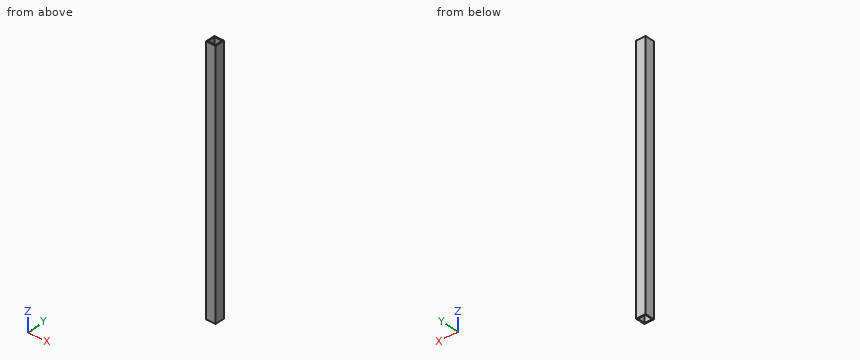
from build123d import *

# Parameters (mm, degrees)
SKETCH1_W           = 30
SKETCH1_H           = 30
SKETCH1_W_2         = 24
SKETCH1_H_2         = 24
BOSS_EXTRUDE2_DEPTH = 784


with BuildPart() as part:
    # Sketch1 → Boss-Extrude2 (new body)
    with BuildSketch(Plane.XY):
        with Locations((-1.115384615, 0.846363591)):
            Rectangle(SKETCH1_W, SKETCH1_H)
        with Locations((-1.115384615, 0.846363591)):
            Rectangle(SKETCH1_W_2, SKETCH1_H_2, mode=Mode.SUBTRACT)
    extrude(amount=BOSS_EXTRUDE2_DEPTH)


solid = part.part
Build history of the part. All positions in model axes, mm. Coordinates: 2 decimals unless noted, no trailing zeros. Write each loop counter-clockwise with the first axis right and the second up, starting at its lowest first coordinate (ties: lowest second). Pieces come first, ordered by that corner, then holes.
(1) Cut at A-A on y = 5.5. List the corners of the cut face in (x, z).
(2) Drill centre lines: line 1 (X direction, y = 0, z = 67); line 2 (Y direction, x = -0.25, z = 61.5). Where is each one in solid material? Low to high.
(3) Pin check, flat tips, straight feed: pin 1 Ø1.5 at (x, y) = (-6, -8.5) entering from -Z; pin 2 Ø12 at (x, y) = (2, 8.5) entering from -Z. Stop position of each tip, or through.
(4) Cut at B-B on x = -1.25. List the corners of the cut face in (y, z).
(5) Cut at C-C on z = 507. List the corners of the cut face in (x, y).
Working result:
1. outline: (-16.12, 0) - (-13.12, 0) - (-13.12, 784) - (-16.12, 784) - close; (10.88, 0) - (13.88, 0) - (13.88, 784) - (10.88, 784) - close
2. line 1: x = -16.12 to -13.12, 10.88 to 13.88
2. line 2: y = -14.15 to -11.15, 12.85 to 15.85
3. pin 1: passes through
3. pin 2: stops at z = 0
4. outline: (-14.15, 0) - (-11.15, 0) - (-11.15, 784) - (-14.15, 784) - close; (12.85, 0) - (15.85, 0) - (15.85, 784) - (12.85, 784) - close
5. outline: (-16.12, -14.15) - (13.88, -14.15) - (13.88, 15.85) - (-16.12, 15.85) - close; hole (-13.12, -11.15) - (10.88, -11.15) - (10.88, 12.85) - (-13.12, 12.85) - close
